For this review, take the finished solid that the model builds, in its own axes (mm). Round coordinates to 2 decimals unless told otherwise and drop trailing zeros. Order: outer loops, then holes, each group sorted by start corner. A loop starts at its lowest first (then second) coordinate and runs counter-clockwise, first axis right, second up.
from build123d import *

# Parameters (mm, degrees)
SKETCH_1_W          = 210
SKETCH_1_H          = 280
EXTRUDE_1_DEPTH     = 12
SKETCH_2_R          = 7.75
SKETCH_2_R_2        = 4.5
CUT_EXTRUDE_1_DEPTH = 176.410946067
SKETCH_3_W          = 60
SKETCH_3_H          = 60
CUT_EXTRUDE_2_DEPTH = 176.410946067
FILLET_1_R          = 5
CHAMFER_1_SIZE      = 2
SKETCH_4_R          = 7.5
CUT_EXTRUDE_3_DEPTH = 9
SKETCH_5_R          = 12
CUT_EXTRUDE_4_DEPTH = 5
CHAMFER_2_SIZE      = 0.3
CHAMFER_3_SIZE      = 0.3


with BuildPart() as part:
    # 草图1 → 凸台-拉伸1 (new body)
    with BuildSketch(Plane(origin=(0, 0, 0), x_dir=(1, 0, 0), z_dir=(0, 1, 0))):
        Rectangle(SKETCH_1_W, SKETCH_1_H)
    extrude(amount=EXTRUDE_1_DEPTH)

    # 草图2 → 切除-拉伸1 (cut, through all)
    with BuildSketch(Plane(origin=(0, 12, 0), x_dir=(1, 0, 0), z_dir=(0, 1, 0))):
        with Locations(Location((0, 0, 0), (0, 0, 270))):
            Circle(SKETCH_2_R)
        with Locations(Location((0, -115, 0), (0, 0, 270))):
            Circle(SKETCH_2_R_2)
        with Locations(Location((0, 115, 0), (0, 0, 270))):
            Circle(SKETCH_2_R_2)
    extrude(amount=-CUT_EXTRUDE_1_DEPTH, mode=Mode.SUBTRACT)

    # 草图3 → 切除-拉伸2 (cut, through all)
    with BuildSketch(Plane(origin=(0, 12, 0), x_dir=(1, 0, 0), z_dir=(0, 1, 0))):
        with Locations((-75, -110)):
            Rectangle(SKETCH_3_W, SKETCH_3_H)
        with Locations((-75, 110)):
            Rectangle(SKETCH_3_W, SKETCH_3_H)
        with Locations((75, 110)):
            Rectangle(SKETCH_3_W, SKETCH_3_H)
        with Locations((75, -110)):
            Rectangle(SKETCH_3_W, SKETCH_3_H)
    extrude(amount=-CUT_EXTRUDE_2_DEPTH, mode=Mode.SUBTRACT)

    # 圆角1
    fillet_1_edges = [part.edges().sort_by_distance(p)[0] for p in [
        (-45, 6, 80),
        (-45, 6, -80),
        (45, 6, -80),
        (45, 6, 80),
    ]]
    fillet(fillet_1_edges, radius=FILLET_1_R)

    # 倒角1
    chamfer_1_edges = [part.edges().sort_by_distance(p)[0] for p in [
        (-105, 6, 80),
        (-45, 6, 140),
        (-105, 6, -80),
        (-45, 6, -140),
        (105, 6, -80),
        (45, 6, -140),
        (105, 6, 80),
        (45, 6, 140),
    ]]
    chamfer(chamfer_1_edges, length=CHAMFER_1_SIZE)

    # 草图4 → 切除-拉伸3 (cut)
    with BuildSketch(Plane(origin=(0, 12, 0), x_dir=(1, 0, 0), z_dir=(0, 1, 0))):
        with Locations(Location((0, -115, 0), (0, 0, 270))):
            Circle(SKETCH_4_R)
        with Locations(Location((0, 115, 0), (0, 0, 270))):
            Circle(SKETCH_4_R)
    extrude(amount=-CUT_EXTRUDE_3_DEPTH, mode=Mode.SUBTRACT)

    # 草图5 → 切除-拉伸4 (cut)
    with BuildSketch(Plane(origin=(0, 12, 0), x_dir=(1, 0, 0), z_dir=(0, 1, 0))):
        with Locations(Location((0, 0, 0), (0, 0, 270))):
            Circle(SKETCH_5_R)
    extrude(amount=-CUT_EXTRUDE_4_DEPTH, mode=Mode.SUBTRACT)

    # 倒角2
    chamfer_2_edges = [part.edges().sort_by_distance(p)[0] for p in [
        (76.5, 12, 80),
        (0, 12, 140),
        (105, 12, 0),
        (45, 12, -111.5),
        (0, 12, -140),
        (-76.5, 12, -80),
        (-105, 12, 0),
        (-45, 12, 111.5),
        (44, 12, -139),
        (104, 12, -79),
        (-44, 12, -139),
        (-104, 12, -79),
        (-104, 12, 79),
        (-44, 12, 139),
        (44, 12, 139),
        (104, 12, 79),
        (-45, 12, -111.5),
        (76.5, 12, -80),
        (45, 12, 111.5),
        (-76.5, 12, 80),
        (-46.464466094, 12, -81.464466094),
        (46.464466094, 12, -81.464466094),
        (46.464466094, 12, 81.464466094),
        (-46.464466094, 12, 81.464466094),
    ]]
    chamfer(chamfer_2_edges, length=CHAMFER_2_SIZE)

    # 倒角3
    chamfer_3_edges = [part.edges().sort_by_distance(p)[0] for p in [
        (76.5, 0, 80),
        (105, 0, 0),
        (0, 0, 140),
        (-45, 0, 111.5),
        (-105, 0, 0),
        (-76.5, 0, -80),
        (0, 0, -140),
        (45, 0, -111.5),
        (44, 0, -139),
        (104, 0, -79),
        (-44, 0, -139),
        (-104, 0, -79),
        (-104, 0, 79),
        (-44, 0, 139),
        (44, 0, 139),
        (104, 0, 79),
        (-45, 0, -111.5),
        (76.5, 0, -80),
        (45, 0, 111.5),
        (-76.5, 0, 80),
        (-46.464466094, 0, -81.464466094),
        (46.464466094, 0, -81.464466094),
        (46.464466094, 0, 81.464466094),
        (-46.464466094, 0, 81.464466094),
    ]]
    chamfer(chamfer_3_edges, length=CHAMFER_3_SIZE)


solid = part.part
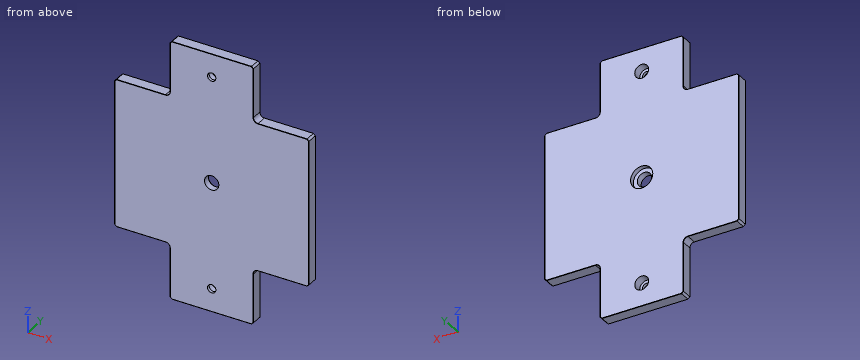
(1) Clearance check with flat-ended pins moving along their axes: P1, Ø5.5, axis at x = -81, y = 7, coming from the +Z side; P2, Ø18, axis at x = 0, z = 0, coming from the +Y side; P3, Ø4, axis at x = 46, y = 5.5, coming from the -Z side; P4, Ø14.5, axis at x = 0, z = 0, coming from the +Y side. State where each tip first meets the part, or that it passes through.
(2) Add section B-B on x = 0. Count the separate pieces of the cut face and the enclosed holes in it, plus the area to 3 significant figures.
(3) Add section C-C on y = 5. Give the boundary of the cut face in (x, z), plus the area to 3 significant figures.
(4) Wall thickness on L1, parallel to X at y = 7.5, z = 115; L2, parallel to X at y = 5.5, z = -121; L3, parallel to Z at x = 54.5, y = 8.5: over which ranges is each line inside the solid? List them lowest first.
(5) Add section D-D on z = -103.5. Give the boundary of the cut face in (x, y).
(6) Add section A-A on z = 0. Give the boundary of the cut face in (x, y).
Here are the results:
1. P1: stops at z = 80
1. P2: stops at y = 7
1. P3: stops at z = -139
1. P4: passes through
2. separate pieces: 4
2. enclosed holes: 0
2. area: 2,810 mm2
3. outline: (-105, -78) - (-103, -80) - (-50, -80) arc R5 cw to (-45, -85) - (-45, -138) - (-43, -140) - (43, -140) - (45, -138) - (45, -85) arc R5 cw to (50, -80) - (103, -80) - (105, -78) - (105, 78) - (103, 80) - (50, 80) arc R5 cw to (45, 85) - (45, 138) - (43, 140) - (-43, 140) - (-45, 138) - (-45, 85) arc R5 cw to (-50, 80) - (-103, 80) - (-105, 78) - close; hole circle Ø15.5 at (0, 0); hole circle Ø15 at (0, -115); hole circle Ø15 at (0, 115)
3. area: 43,900 mm2
4. L1: x = -45 to -7.5, 7.5 to 45
4. L2: x = -45 to -4.5, 4.5 to 45
4. L3: z = -80 to 80
5. outline: (-45, 0.3) - (-44.7, 0) - (44.7, 0) - (45, 0.3) - (45, 11.7) - (44.7, 12) - (-44.7, 12) - (-45, 11.7) - close
6. outline: (-105, 0.3) - (-104.7, 0) - (-7.75, 0) - (-7.75, 7) - (-12, 7) - (-12, 12) - (-104.7, 12) - (-105, 11.7) - close; (7.75, 0) - (104.7, 0) - (105, 0.3) - (105, 11.7) - (104.7, 12) - (12, 12) - (12, 7) - (7.75, 7) - close
